CAD build for the part. Positions are in the model's coordinates, mm. Face numbers are marked on the shaded views. A direction names the side the tool comes from. Round coordinates to 2 decimals unless told otherwise and drop trailing zeros. Order: outer loops, then holes, each group sorted by start corner. A loop starts at its lowest first (then second) coordinate and runs counter-clockwise, first axis right, second up. Notation, with made-up numbers: (74.5, 87.25) -> (92.5, 87.25) arc R20 cw to (92.5, 95.25) -> close; hole circle Ø6 at (3.25, 84.25). An arc over 180 degrees is marked (long way). Return JSON: item names as keys, results as strings. Group by question number.
Q1. Cut at B-B (z = 0). Write the cut outline in (x, y).
Q2. Probe line 1 along Y through (x, z) = (-26.5, 0); line 2 along Z through (x, y) = (-13, 90); line 3 along Y through (x, z) = (15, 0). List the from-to ranges inside material, lowest first.
Q3. Cut at A-A (x = -25). Write the cut outline in (y, z), then the cut area to 3 significant figures.
Q4. Which spindle directions (+Z, -Z, +X, -X, +Y, -Y) get a long thin tool onto all of the face, cutting with end or side? Do the marked faces 4, 5 and 6. Say none if no direction does.
Q5. Cut at D-D (z = 49). Write the cut outline in (x, y).
Q6. Flat gauge pins, fed straight in: pin 1 (8 mm diameter, centred on x = -19, y = 54, fed in from -Z); pin 2 (6 mm diameter, centred on x = 25.5, z = 46, fed in from +Y); pin 3 (1 mm diameter, centred on y = 145.5, z = -35.5, fed in from -X); pin 4 (5 mm diameter, centred on x = -33, z = 12.5, fed in from -Y). Where does each tip first touch, or does it go through?
Q7. Cut at C-C (y = 232.5). Write the cut outline in (x, z), then the cut area to 3 significant figures.
Q8. Mould opens along Y. For the marked faces 1, 2 and 3 say: +Y half, -Y half, draft (parallel to the pull), parting line (faces both ways), or undercut.
from build123d import *

# Parameters (mm, degrees)
BASE_PLATE_SKETCH_W         = 210
BASE_PLATE_SKETCH_H         = 115
BASE_PLATE_210X115X30_DEPTH = 30
PEDESTAL_SKETCH_W           = 100
PEDESTAL_SKETCH_H           = 60
PEDESTAL_100X60X32_DEPTH    = 32
PEDESTAL_FILLET_R20_R       = 20
CLAMP_BLOCK_DEPTH           = 57.5
CROSS_HOLES_SKETCH_R        = 15
CROSS_HOLES_2X_30_DEPTH     = 115
CLAMP_BAND_DEPTH            = 100


with BuildPart() as part:
    # Base Plate Sketch → Base Plate 210x115x30 (new body)
    with BuildSketch(Plane(origin=(0, 0, 0), x_dir=(1, 0, 0), z_dir=(0, 1, 0))):
        Rectangle(BASE_PLATE_SKETCH_W, BASE_PLATE_SKETCH_H)
    extrude(amount=BASE_PLATE_210X115X30_DEPTH)

    # Pedestal Sketch → Pedestal 100x60x32 (add)
    with BuildSketch(Plane(origin=(0, 30, 0), x_dir=(1, 0, 0), z_dir=(0, 1, 0))):
        Rectangle(PEDESTAL_SKETCH_W, PEDESTAL_SKETCH_H)
    extrude(amount=PEDESTAL_100X60X32_DEPTH)

    # Pedestal Fillet R20
    pedestal_fillet_r20_edges = [part.edges().sort_by_distance(p)[0] for p in [
        (50, 30, 0),
        (-50, 30, 0),
    ]]
    fillet(pedestal_fillet_r20_edges, radius=PEDESTAL_FILLET_R20_R)

    # Clamp Block Profile Sketch → Clamp Block (add, symmetric)
    with BuildSketch(Plane.XY):
        with BuildLine():
            Line((50, 62), (50, 118))
            Line((50, 118), (50, 135.5))
            Line((50, 135.5), (58, 135.5))
            Line((58, 135.5), (58, 180.5))
            Line((58, 180.5), (50, 180.5))
            Line((50, 180.5), (50, 198))
            Line((50, 198), (50, 268))
            Line((50, 268), (-50, 268))
            Line((-50, 268), (-50, 198))
            Line((-50, 198), (10, 198))
            ThreePointArc((10, 198), (50, 158), (10, 118))
            Line((10, 118), (-50, 118))
            Line((-50, 118), (-50, 62))
            Line((-50, 62), (50, 62))
        make_face()
    extrude(amount=CLAMP_BLOCK_DEPTH, both=True)

    # Cross Holes Sketch → Cross Holes 2xØ30 (cut)
    with BuildSketch(Plane.ZY.offset(50)):
        with Locations((0, 90.5)):
            Circle(CROSS_HOLES_SKETCH_R)
        with Locations((0, 232.5)):
            Circle(CROSS_HOLES_SKETCH_R)
    extrude(amount=-CROSS_HOLES_2X_30_DEPTH, mode=Mode.SUBTRACT)

    # Clamp Band Sketch → Clamp Band (add)
    with BuildSketch(Plane.ZY.offset(50)):
        with BuildLine():
            Line((-57.5, 268), (57.5, 268))
            ThreePointArc((57.5, 268), (0, 283.407078565), (-57.5, 268))
        make_face()
    extrude(amount=-CLAMP_BAND_DEPTH)


solid = part.part
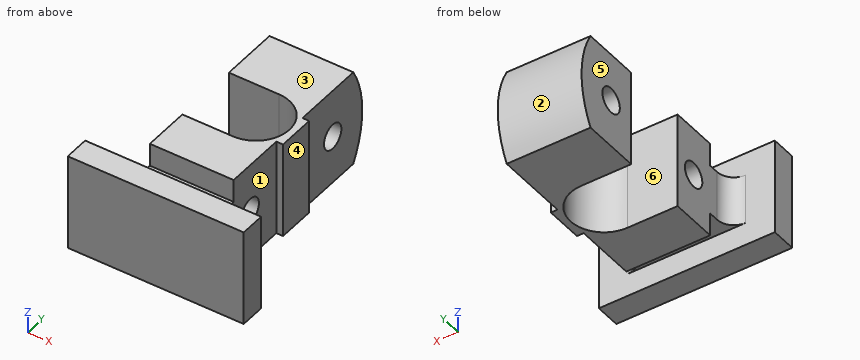
Solution:
{
 "1": {"outline": "(-105, 0) -> (105, 0) -> (105, 30) -> (70, 30) arc R20 cw to (50, 50) -> (50, 75.5) -> (-50, 75.5) -> (-50, 50) arc R20 cw to (-70, 30) -> (-105, 30) -> close; (-50, 105.5) -> (50, 105.5) -> (50, 135.5) -> (58, 135.5) -> (58, 180.5) -> (50, 180.5) -> (50, 217.5) -> (-50, 217.5) -> (-50, 198) -> (10, 198) arc R40 cw to (10, 118) -> (-50, 118) -> close; (-50, 247.5) -> (50, 247.5) -> (50, 283.41) -> (-50, 283.41) -> close"},
 "2": {"line 1": "y = 0 to 75.5, 105.5 to 118, 198 to 217.5, 247.5 to 283.41", "line 2": "z = -57.5 to -14.99, 14.99 to 57.5", "line 3": "y = 0 to 75.5, 105.5 to 118.31, 197.69 to 217.5, 247.5 to 283.41"},
 "3": {"outline": "(0, -57.5) -> (30, -57.5) -> (30, -30) -> (62, -30) -> (62, -57.5) -> (118, -57.5) -> (118, 57.5) -> (62, 57.5) -> (62, 30) -> (30, 30) -> (30, 57.5) -> (0, 57.5) -> close; (198, -57.5) -> (268, -57.5) arc R115 ccw to (268, 57.5) -> (198, 57.5) -> close; hole circle Ø30 at (90.5, 0); hole circle Ø30 at (232.5, 0)", "area": "19,600 mm²"},
 "4": {"face 4": "+Z, -Z, +X, +Y", "face 5": "+Z, -Z, -X, +Y", "face 6": "+Z, -Z, -X"},
 "5": {"outline": "(-105, 0) -> (105, 0) -> (105, 30) -> (-105, 30) -> close; (-50, 62) -> (50, 62) -> (50, 135.5) -> (58, 135.5) -> (58, 180.5) -> (50, 180.5) -> (50, 272.45) -> (-50, 272.45) -> (-50, 198) -> (10, 198) arc R40 cw to (10, 118) -> (-50, 118) -> close"},
 "6": {"pin 1": "stops at z = -30", "pin 2": "stops at y = 275.07", "pin 3": "stops at x = 47.83", "pin 4": "stops at y = 0"},
 "7": {"outline": "(-50, -57.5) -> (50, -57.5) -> (50, -15) -> (-50, -15) -> close; (-50, 15) -> (50, 15) -> (50, 57.5) -> (-50, 57.5) -> close", "area": "8,500 mm²"},
 "8": {"face 1": "undercut", "face 2": "+Y half", "face 3": "draft"}
}
